from build123d import *

# Parameters (mm, degrees)
SKETCH1_W           = 150
SKETCH1_H           = 300
SKETCH1_R           = 9
BOSS_EXTRUDE1_DEPTH = 10


with BuildPart() as part:
    # Sketch1 → Boss-Extrude1 (new body)
    with BuildSketch(Plane.XY):
        Rectangle(SKETCH1_W, SKETCH1_H)
        with Locations((-45, 100)):
            Circle(SKETCH1_R, mode=Mode.SUBTRACT)
        with Locations((-45, 0)):
            Circle(SKETCH1_R, mode=Mode.SUBTRACT)
        with Locations((-45, -100)):
            Circle(SKETCH1_R, mode=Mode.SUBTRACT)
        with Locations(Location((45, -100, 0), (0, 0, 180))):
            Circle(SKETCH1_R, mode=Mode.SUBTRACT)
        with Locations(Location((45, 0, 0), (0, 0, 180))):
            Circle(SKETCH1_R, mode=Mode.SUBTRACT)
        with Locations(Location((45, 100, 0), (0, 0, 180))):
            Circle(SKETCH1_R, mode=Mode.SUBTRACT)
    extrude(amount=BOSS_EXTRUDE1_DEPTH)


solid = part.part
For this review, take the finished solid that the model builds, in its own axes (mm). Round coordinates to 2 decimals unless told otherwise and drop trailing zeros. Loops run counter-clockwise (first coordinate to the right, second up) from the corner with the lowest first, then second, coordinate; pieces in that order, holes last. Notation, with made-up numbers: (-36.75, -17) - (-6.75, -17) arc R22 ccw to (-6.75, 9) - close; hole circle Ø2 at (-38.75, 33). An arc over 180 degrees is marked (long way). One line per question, with ' | ' between items.
Q1. For line 1 along Y through (x, z) = (45, 7); line 2 along X through (y, z) = (2, 9); line 3 along Y through (x, z) = (-42, 6), list the stretches that pass through material, from the lowest coordinate up. Write a range as [from, to].
Taken from the geometry:
line 1: y = [-150, -109], [-91, -9], [9, 91], [109, 150] | line 2: x = [-75, -53.77], [-36.23, 36.23], [53.77, 75] | line 3: y = [-150, -108.49], [-91.51, -8.49], [8.49, 91.51], [108.49, 150]
Q2. Take a section at A-A (z = 5.25). Give the boundary of the cut face in (x, y), and give its area (3 significant figures).
Taken from the geometry:
outline: (-75, -150) - (75, -150) - (75, 150) - (-75, 150) - close; hole circle Ø18 at (-45, -100); hole circle Ø18 at (-45, 0); hole circle Ø18 at (-45, 100); hole circle Ø18 at (45, -100); hole circle Ø18 at (45, 0); hole circle Ø18 at (45, 100) | area: 43,500 mm²
Q3. The part is to be moulded in two halves that separate along Y. For faces 1 (the flat face through (-1, 150, 5)), 2 (the flat face through (-1, 2, 0)), 3 (the cylindrical face through (46.951, -91.214, 4.93)), say which applies: released by +Y, released by -Y, zero draft, split by the parting line, or undercut.
Taken from the geometry:
face 1: released by +Y | face 2: zero draft | face 3: undercut
Q4. Take a section at B-B (y = -100). Give the boundary of the cut face in (x, z), and give its area (3 significant figures).
Taken from the geometry:
outline: (-75, 0) - (-54, 0) - (-54, 10) - (-75, 10) - close; (-36, 0) - (36, 0) - (36, 10) - (-36, 10) - close; (54, 0) - (75, 0) - (75, 10) - (54, 10) - close | area: 1,140 mm²
Q5. Take a section at C-C (x = 45). Give the boundary of the cut face in (y, z).
Taken from the geometry:
outline: (-150, 0) - (-109, 0) - (-109, 10) - (-150, 10) - close; (-91, 0) - (-9, 0) - (-9, 10) - (-91, 10) - close; (9, 0) - (91, 0) - (91, 10) - (9, 10) - close; (109, 0) - (150, 0) - (150, 10) - (109, 10) - close
